from build123d import *

# Parameters (mm, degrees)
CHAMFER1_SIZE              = 1
CUT_EXTRUDE1_DEPTH         = 55.911039474
CUT_EXTRUDE1_DEPTH_BACK    = 55.911039474
SKETCH3_W                  = 1
SKETCH3_H                  = 15
M14X1_5_TAPPED_HOLE1_D     = 12.5
M14X1_5_TAPPED_HOLE1_DEPTH = 20
M14X1_5_TAPPED_HOLE1_TIP   = 3.755378869


with BuildPart() as part:
    # Sketch2 → Revolve1 (revolve)
    with BuildSketch(Plane.XY, mode=Mode.PRIVATE) as revolve1_sk:
        Polygon((0, 48.654108317), (-18, 48.654108317), (-18, 33.654108317), (-12, 33.654108317), (-12, -21.345891683), (0, -21.345891683), align=None)
    revolve(revolve1_sk.sketch.rotate(Axis((0, 14.106387272, 0), (0, -1, 0)), 270), axis=Axis((0, 14.106387272, 0), (0, -1, 0)))

    # Chamfer1
    chamfer1_edges = [part.edges().sort_by_distance(p)[0] for p in [
        (0, -21.345891683, -12),
        (0, 33.654108317, -18),
        (0, 48.654108317, -18),
    ]]
    chamfer(chamfer1_edges, length=CHAMFER1_SIZE)

    # Sketch3 → Cut-Extrude1 (cut, two sides: drawn at the far end of the back side and taken through both)
    with BuildSketch(Plane.XY.offset(-CUT_EXTRUDE1_DEPTH_BACK)):
        with Locations((-11.5, -8.845891683)):
            Rectangle(SKETCH3_W, SKETCH3_H)
        with Locations((11.5, -8.845891683)):
            Rectangle(SKETCH3_W, SKETCH3_H)
    extrude(amount=CUT_EXTRUDE1_DEPTH + CUT_EXTRUDE1_DEPTH_BACK, mode=Mode.SUBTRACT)

    # M14x1.5 Tapped Hole1
    with Locations(Plane(origin=(0, -21.345891683, 0), x_dir=(-1, 0, 0), z_dir=(0, -1, 0))):
        with Locations((0, 0)):
            Hole(M14X1_5_TAPPED_HOLE1_D / 2, depth=M14X1_5_TAPPED_HOLE1_DEPTH)
            with Locations((0, 0, -(M14X1_5_TAPPED_HOLE1_DEPTH + M14X1_5_TAPPED_HOLE1_TIP / 2))):  # 118° drill point
                Cone(0, M14X1_5_TAPPED_HOLE1_D / 2, M14X1_5_TAPPED_HOLE1_TIP, mode=Mode.SUBTRACT)


solid = part.part
Source: CAD feature listing. Evaluate the final solid. Frame: model axes, mm. A direction names the side the tool comes from. Give positions to 0.01 mm unless a question says otherwise; leave off trailing zeros. Write each loop counter-clockwise with the first axis right and the second up, starting at its lowest first coordinate (ties: lowest second). Pieces come first, ordered by that corner, then holes. Notation, with made-up numbers: (35.5, 17.25) -> (94.5, 17.25) arc R19 ccw to (94.5, 25.25) -> close; hole circle Ø8 at (75, 23). An arc over 180 degrees is marked (long way). Return JSON: item names as keys, results as strings. Group by question number.
1. Mould query, pull axis Z, two halves, no side actions, for faces 1 (the face through (11, -9, 0)), 2 (the face through (-1.035, 1.757, -0.326)), 3 (the face through (4.596, 6.276, 11.085)), 4 (the face through (5.96, -11.21, -1.88)). Classes: +Z half, -Z half, draft (parallel to the pull), parting line (faces both ways), or undercut.
2. Pin query (flat end, axial travel): pin 1 Ø2 at (x, y) = (-9, -13.5) entering from -Z; pin 2 Ø1 at (x, y) = (1, 12) entering from +Z; pin 3 Ø4 at (y, z) = (17.5, -12) entering from +X. Return the tip coordinate at first contact, or that it passes through.
3. Material intervals for line 1 (Y direction, x = -6.5, z = -11); line 2 (X direction, y = 5, z = 0); line 3 (Z direction, x = -1, y = -10), sorted ascending. Write a range as from..to.
4. Section A-A, the plane y = 35.5. Output: boundary loops of the cut face in (x, z).
5. Access query for faces 5 (the face through (-5.407, 41.063, 17.169)), 6 (the face through (4, 33.654, -12)), 7 (the face through (-11, -9, 0)). Directions: +Z, -Z, +X, -X, +Y, -Y. A direction counts if a zero-diameter tool reaches every point of the face in a straight line with its end or side. Return the directions, or none.
Determined:
{
 "1": {"face 1": "draft", "face 2": "undercut", "face 3": "parting line", "face 4": "undercut"},
 "2": {"pin 1": "stops at z = -8.94", "pin 2": "stops at z = 11.99", "pin 3": "stops at x = 6.63"},
 "3": {"line 1": "y = 33.65..48.65", "line 2": "x = -12..12", "line 3": "z = -11.96..-6.17, 6.17..11.96"},
 "4": {"outline": "circle Ø36 at (0, 0)"},
 "5": {"face 5": "+Y, -Y", "face 6": "-Y", "face 7": "+Z, -Z, -X"}
}
